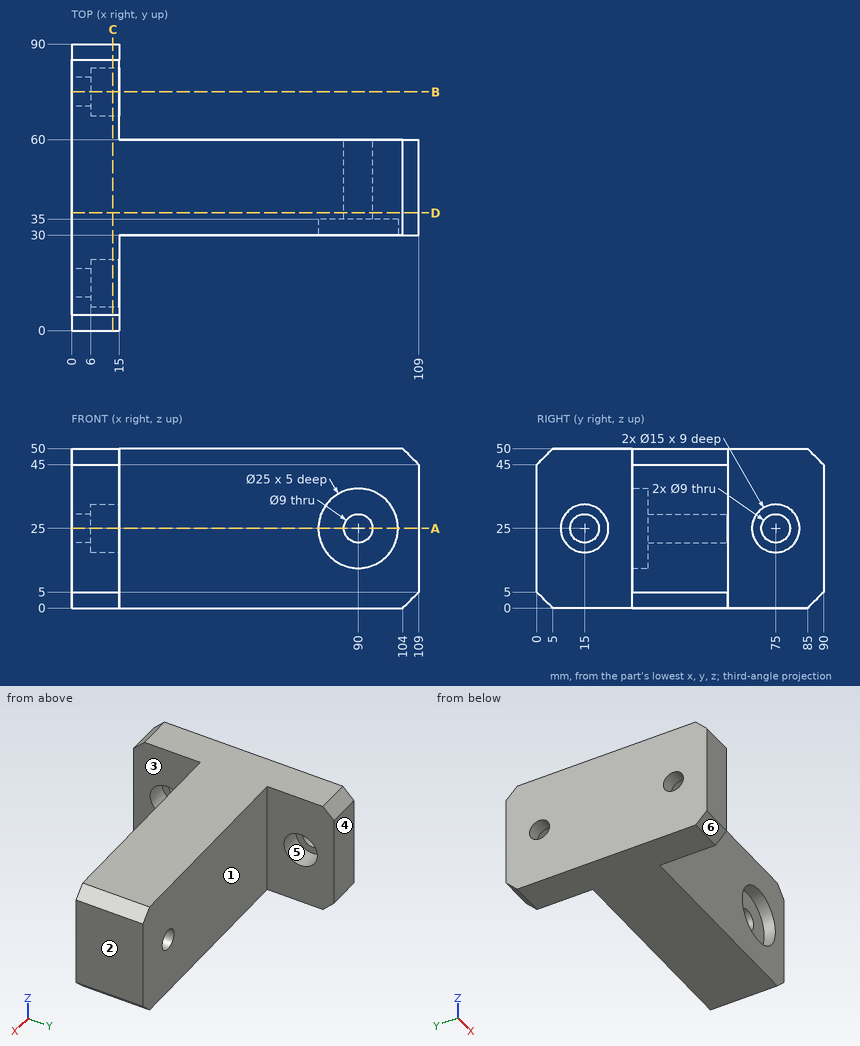
Check sheet for the drawn part. Datum: minimum x, y, z corner. Units: mm. A direction names the side the tool comes from. Round coordinates to 2 decimals unless told otherwise and drop trailing zeros. Order: outer loops, then holes, each group sorted by start corner. A loop starts at its lowest first (then second) coordinate and runs counter-clockwise, first axis right, second up.
(1) Access from +Z, -Z, +X, -X, +Y, -Y to the whole of each face (thin tool, end or side, straight path). Record for the marked faces 1, 2 and 3.
(2) Cross-section at A-A, the plane z = 25. State how many separate pieces and enclosed holes the cut face has, and give its area (3 significant figures).
(3) Cross-section at B-B, the plane y = 75. Enter the section's corners in (x, z).
(4) Scan lines: probe 1 along Y at (x, z) = (2.45, 25); probe 2 along Y at (x, z) = (8.75, 25); probe 3 along X at (y, z) = (33.2, 25). Record each from-to range of solid material in increasing order.
(5) Draft check along Y on the marked faces 4, 5 and 6. Enter one of: pulls with the +Y half, pulls with the -Y half, needs draft (parallel to the pull), parting line crosses it, or undercut.
(6) Go/stop test with flat-tipped pins: P1, Ø15, axis at y = 71.5, z = 37, coming from the +X side; P2, Ø8, axis at x = 48.5, z = 26.5, coming from the -Y side; P3, Ø1.5, axis at x = 39, z = 36.5, coming from the +Y side. Record where each tip stops, or that it passes through.
(7) Cross-section at C-C, the plane x = 13. Enter the section's corners in (y, z), and give its area (3 significant figures).
(8) Cross-section at D-D, the plane y = 37. Enter the section's corners in (x, z).
Check sheet entries:
1. face 1: +Z, -Z, +X, +Y
1. face 2: +Z, -Z, +X, +Y, -Y
1. face 3: +Z, -Z, +X, -Y
2. separate pieces: 4
2. enclosed holes: 0
2. area: 3,440 mm2
3. outline: (0, 0) - (15, 0) - (15, 17.5) - (6, 17.5) - (6, 20.5) - (0, 20.5) - close; (0, 29.5) - (6, 29.5) - (6, 32.5) - (15, 32.5) - (15, 50) - (0, 50) - close
4. probe 1: y = 0 to 10.5, 19.5 to 70.5, 79.5 to 90
4. probe 2: y = 0 to 7.5, 22.5 to 67.5, 82.5 to 90
4. probe 3: x = 0 to 77.5, 102.5 to 109
5. face 4: pulls with the +Y half
5. face 5: undercut
5. face 6: pulls with the -Y half
6. P1: stops at x = 15
6. P2: stops at y = 30
6. P3: stops at y = 60
7. outline: (0, 5) - (5, 0) - (85, 0) - (90, 5) - (90, 45) - (85, 50) - (5, 50) - (0, 45) - close; hole circle Ø15 at (15, 25); hole circle Ø15 at (75, 25)
7. area: 4,100 mm2
8. outline: (0, 0) - (104, 0) - (109, 5) - (109, 45) - (104, 50) - (0, 50) - close; hole circle Ø9 at (90, 25)
